from build123d import *

# Parameters (mm, degrees)
BOSS_EXTRUDE1_DEPTH     = 24
CUT_EXTRUDE2_DEPTH      = 39.742741256
CUT_EXTRUDE2_DEPTH_BACK = 39.742741256
SKETCH4_R               = 2
CUT_EXTRUDE3_DEPTH      = 39.742741256
CUT_EXTRUDE3_DEPTH_BACK = 39.742741256
SKETCH6_W               = 32.588779774
SKETCH6_H               = 20
SKETCH7_R               = 2
CUT_EXTRUDE4_DEPTH      = 39.742741256
SKETCH8_R               = 1.5
BOSS_EXTRUDE3_DEPTH     = 22


with BuildPart() as part:
    # Sketch1 → Boss-Extrude1 (new body)
    with BuildSketch(Plane(origin=(0, 0, 0), x_dir=(1, 0, 0), z_dir=(0, 1, 0))):
        with BuildLine():
            Line((-5, 0), (-5, -30))
            Line((-5, -30), (5, -30))
            Line((5, -30), (5, 0))
            ThreePointArc((5, 0), (0, 5), (-5, 0))
        make_face()
    extrude(amount=BOSS_EXTRUDE1_DEPTH)

    # Sketch4 → Cut-Extrude2 (cut, two sides: drawn at the far end of the back side and taken through both)
    with BuildSketch(Plane(origin=(0, 24, 0), x_dir=(1, 0, 0), z_dir=(0, 1, 0)).offset(-CUT_EXTRUDE2_DEPTH_BACK)):
        with Locations(Location((0, 0, 0), (0, 0, 270))):
            Circle(SKETCH4_R)
    extrude(amount=CUT_EXTRUDE2_DEPTH + CUT_EXTRUDE2_DEPTH_BACK, mode=Mode.SUBTRACT)

    # Sketch6 → Cut-Extrude3 (cut, two sides: drawn at the far end of the back side and taken through both)
    with BuildSketch(Plane(origin=(0, 0, 0), x_dir=(0, 0, -1), z_dir=(1, 0, 0)).offset(-CUT_EXTRUDE3_DEPTH_BACK)):
        with Locations((-8.705610113, 12)):
            Rectangle(SKETCH6_W, SKETCH6_H)
    extrude(amount=CUT_EXTRUDE3_DEPTH + CUT_EXTRUDE3_DEPTH_BACK, mode=Mode.SUBTRACT)

    # Sketch7 → Cut-Extrude4 (cut, through all)
    with BuildSketch(Plane(origin=(0, 0, 25), x_dir=(-1, 0, 0), z_dir=(0, 0, -1))):
        with Locations(Location((0, 12, 0), (0, 0, 90))):
            Circle(SKETCH7_R)
    extrude(amount=-CUT_EXTRUDE4_DEPTH, mode=Mode.SUBTRACT)

    # Sketch8 → Boss-Extrude3 (add)
    with BuildSketch(Plane(origin=(0, 24, 0), x_dir=(1, 0, 0), z_dir=(0, 1, 0))):
        with Locations(Location((-2, -8, 0), (0, 0, 270))):
            Circle(SKETCH8_R)
        with Locations(Location((2, -14, 0), (0, 0, 270))):
            Circle(SKETCH8_R)
    extrude(amount=-BOSS_EXTRUDE3_DEPTH)


solid = part.part
The model under review builds one solid part; all positions refer to its coordinate system, in mm. A direction names the side the tool comes from. Round coordinates to 2 decimals unless told otherwise and drop trailing zeros. Loops run counter-clockwise (first coordinate to the right, second up) from the corner with the lowest first, then second, coordinate; pieces in that order, holes last. Notation, with made-up numbers: (-22, 87) -> (5, 87) arc R21 cw to (5, 124) -> close; hole circle Ø6 at (19.5, -25.75). An arc over 180 degrees is marked (long way). Write item = value, one per line. Start each with the question number.
Item 1: Take a section at C-C on z = 20.5. Give the boundary of the cut face in (x, y), plus the area to 3 significant figures.
Item 2: Take a section at B-B on z = 1. Give the boundary of the cut face in (x, y).
Item 3: Mouldability with a two-part tool opening along Z and no side actions: class faces 4 (the flat face through (0, 24, 12)), 5 (the flat face through (0, 2, 10)), 6 (the cylindrical face through (0, 1, -5)) as released by +Z, released by -Z, zero draft, split by the parting line, or undercut.
Item 4: For faces 1 (the flat face through (2.2, 11.9, 25)), 2 (the cylindrical face through (-1.2, 10.4, 27.5)), 3 (the cylindrical face through (2.07, 12.14, 12.5)), list the 3-axis set-ups (+Z, -Z, +X, -X, +Y, -Y) from which the entire face can be reached by the end or side of a thin tool; tool diameter is ignored.
Item 5: Insertion check: pin 1 (6 mm diameter, centred on y = 16.5, z = 13.5, fed in from +X). The pin has a flat end and moves straight along its axis. Give the tip position at first contact, or say it passes through.
Item 6: To check wall thickness, follow L1, parallel to Y at x = -2.75, z = 17.5; L2, parallel to Z at x = 0, y = 0.4; L3, parallel to X at y = 12, z = 29. State the ranges of each line that lie inside material, in increasing order.
Item 7: Take a section at A-A on y = 12. Give the boundary of the cut face in (x, z).
Item 8: Take a section at D-D on x = -2.5. Give the boundary of the cut face in (y, z).
Result:
q1.outline = (-5, 0) -> (5, 0) -> (5, 2) -> (-5, 2) -> close; (-5, 22) -> (5, 22) -> (5, 24) -> (-5, 24) -> close
q1.area = 40.0 mm²
q2.outline = (-5, 0) -> (-1.73, 0) -> (-1.73, 2) -> (-5, 2) -> close; (-5, 22) -> (-1.73, 22) -> (-1.73, 24) -> (-5, 24) -> close; (1.73, 0) -> (5, 0) -> (5, 2) -> (1.73, 2) -> close; (1.73, 22) -> (5, 22) -> (5, 24) -> (1.73, 24) -> close
q3.face_4 = zero draft
q3.face_5 = undercut
q3.face_6 = released by -Z
q4.face_1 = +X, -X
q4.face_2 = +Z
q4.face_3 = none
q5.pin_1 = 3.5
q6.L1 = 0 to 2, 22 to 24
q6.L2 = -5 to -2, 2 to 30
q6.L3 = -5 to -2, 2 to 5
q7.outline = (-5, 25) -> (-2, 25) -> (-2, 30) -> (-5, 30) -> close; circle Ø3 at (-2, 8); circle Ø3 at (2, 14); (2, 25) -> (5, 25) -> (5, 30) -> (2, 30) -> close
q8.outline = (0, -4.33) -> (2, -4.33) -> (2, 6.59) -> (22, 6.59) -> (22, -4.33) -> (24, -4.33) -> (24, 30) -> (0, 30) -> close; hole (2, 9.41) -> (22, 9.41) -> (22, 25) -> (2, 25) -> close
